from build123d import *

# Parameters (mm, degrees)
ELBOW_SECTION_SKETCH_210_290_R    = 145
ELBOW_SECTION_SKETCH_210_290_R_2  = 105
FLANGE_A_SKETCH_R                 = 105
FLANGE_A_360X360X50_DEPTH         = 50
FLANGE_START                      = -50
FLANGE_B_SKETCH_R                 = 105
FLANGE_B_360X360X50_DEPTH         = 50
EDGE_CHAMFER_5X45_A_SIZE          = 5
EDGE_CHAMFER_5X45_B_SIZE          = 5
FLANGE_B_BOLT_HOLES_SKETCH_R      = 15
FLANGE_B_BOLT_HOLES_30_DEPTH      = 50
FLANGE_B_COUNTERBORES_SKETCH_R    = 30
FLANGE_B_COUNTERBORES_60X10_DEPTH = 10
FLANGE_A_BOLT_HOLES_SKETCH_R      = 15
FLANGE_A_BOLT_HOLES_30_DEPTH      = 50
FLANGE_A_COUNTERBORES_SKETCH_R    = 30
FLANGE_A_COUNTERBORES_60X10_DEPTH = 10


with BuildPart() as part:
    # Elbow Body: sweep along a path in Elbow Path Sketch
    with BuildLine(Plane.XY) as elbow_body_path:
        Line((0, 0), (0, 150))
        ThreePointArc((0, 150), (76.152236891, 333.847763109), (260, 410))
        Line((260, 410), (410, 410))
    # Elbow Section Sketch Ø210-Ø290 → Elbow Body (sweep)
    with BuildSketch(Plane(origin=(410, 0, 0), x_dir=(0, 0, -1), z_dir=(1, 0, 0))):
        with Locations((0, 410)):
            Circle(ELBOW_SECTION_SKETCH_210_290_R)
        with Locations((0, 410)):
            Circle(ELBOW_SECTION_SKETCH_210_290_R_2, mode=Mode.SUBTRACT)
    sweep(path=elbow_body_path.line)

    # Flange A Sketch → Flange A 360x360x50 (add)
    with BuildSketch(Plane(origin=(410, 0, 0), x_dir=(0, 0, -1), z_dir=(1, 0, 0))):
        with BuildLine():
            Line((-160, 230), (160, 230))
            ThreePointArc((160, 230), (174.142135624, 235.857864376), (180, 250))
            Line((180, 250), (180, 570))
            ThreePointArc((180, 570), (174.142135624, 584.142135624), (160, 590))
            Line((160, 590), (-160, 590))
            ThreePointArc((-160, 590), (-174.142135624, 584.142135624), (-180, 570))
            Line((-180, 570), (-180, 250))
            ThreePointArc((-180, 250), (-174.142135624, 235.857864376), (-160, 230))
        make_face()
        with Locations((0, 410)):
            Circle(FLANGE_A_SKETCH_R, mode=Mode.SUBTRACT)
    extrude(amount=-FLANGE_A_360X360X50_DEPTH)

    # Flange B Sketch → Flange B 360x360x50 (add)
    with BuildSketch(Plane.XZ.offset(FLANGE_START)):
        with BuildLine():
            Line((-160, -180), (160, -180))
            ThreePointArc((160, -180), (174.142135624, -174.142135624), (180, -160))
            Line((180, -160), (180, 160))
            ThreePointArc((180, 160), (174.142135624, 174.142135624), (160, 180))
            Line((160, 180), (-160, 180))
            ThreePointArc((-160, 180), (-174.142135624, 174.142135624), (-180, 160))
            Line((-180, 160), (-180, -160))
            ThreePointArc((-180, -160), (-174.142135624, -174.142135624), (-160, -180))
        make_face()
        with Locations(Location((0, 0, 0), (0, 0, 180))):
            Circle(FLANGE_B_SKETCH_R, mode=Mode.SUBTRACT)
    extrude(amount=FLANGE_B_360X360X50_DEPTH)

    # Edge Chamfer 5x45 A
    edge_chamfer_5x45_a_edges = [part.edges().sort_by_distance(p)[0] for p in [
        (0, 0, 105),
    ]]
    chamfer(edge_chamfer_5x45_a_edges, length=EDGE_CHAMFER_5X45_A_SIZE)

    # Edge Chamfer 5x45 B
    edge_chamfer_5x45_b_edges = [part.edges().sort_by_distance(p)[0] for p in [
        (410, 410, 105),
    ]]
    chamfer(edge_chamfer_5x45_b_edges, length=EDGE_CHAMFER_5X45_B_SIZE)

    # Flange B Bolt Holes Sketch → Flange B Bolt Holes Ø30 (cut)
    with BuildSketch(Plane.XZ):
        with Locations(Location((-130, 130, 0), (0, 0, 270))):
            Circle(FLANGE_B_BOLT_HOLES_SKETCH_R)
        with Locations(Location((-130, -130, 0), (0, 0, 270))):
            Circle(FLANGE_B_BOLT_HOLES_SKETCH_R)
        with Locations(Location((130, -130, 0), (0, 0, 90))):
            Circle(FLANGE_B_BOLT_HOLES_SKETCH_R)
        with Locations(Location((130, 130, 0), (0, 0, 90))):
            Circle(FLANGE_B_BOLT_HOLES_SKETCH_R)
    extrude(amount=-FLANGE_B_BOLT_HOLES_30_DEPTH, mode=Mode.SUBTRACT)

    # Flange B Counterbores Sketch → Flange B Counterbores Ø60x10 (cut)
    with BuildSketch(Plane.XZ):
        with Locations(Location((-130, 130, 0), (0, 0, 270))):
            Circle(FLANGE_B_COUNTERBORES_SKETCH_R)
        with Locations(Location((-130, -130, 0), (0, 0, 270))):
            Circle(FLANGE_B_COUNTERBORES_SKETCH_R)
        with Locations(Location((130, -130, 0), (0, 0, 270))):
            Circle(FLANGE_B_COUNTERBORES_SKETCH_R)
        with Locations(Location((130, 130, 0), (0, 0, 270))):
            Circle(FLANGE_B_COUNTERBORES_SKETCH_R)
    extrude(amount=-FLANGE_B_COUNTERBORES_60X10_DEPTH, mode=Mode.SUBTRACT)

    # Flange A Bolt Holes Sketch → Flange A Bolt Holes Ø30 (cut)
    with BuildSketch(Plane(origin=(410, 0, 0), x_dir=(0, 0, -1), z_dir=(1, 0, 0))):
        with Locations((-130, 540)):
            Circle(FLANGE_A_BOLT_HOLES_SKETCH_R)
        with Locations((-130, 280)):
            Circle(FLANGE_A_BOLT_HOLES_SKETCH_R)
        with Locations(Location((130, 280, 0), (0, 0, 180))):
            Circle(FLANGE_A_BOLT_HOLES_SKETCH_R)
        with Locations(Location((130, 540, 0), (0, 0, 180))):
            Circle(FLANGE_A_BOLT_HOLES_SKETCH_R)
    extrude(amount=-FLANGE_A_BOLT_HOLES_30_DEPTH, mode=Mode.SUBTRACT)

    # Flange A Counterbores Sketch → Flange A Counterbores Ø60x10 (cut)
    with BuildSketch(Plane(origin=(410, 0, 0), x_dir=(0, 0, -1), z_dir=(1, 0, 0))):
        with Locations((-130, 540)):
            Circle(FLANGE_A_COUNTERBORES_SKETCH_R)
        with Locations((130, 540)):
            Circle(FLANGE_A_COUNTERBORES_SKETCH_R)
        with Locations((-130, 280)):
            Circle(FLANGE_A_COUNTERBORES_SKETCH_R)
        with Locations((130, 280)):
            Circle(FLANGE_A_COUNTERBORES_SKETCH_R)
    extrude(amount=-FLANGE_A_COUNTERBORES_60X10_DEPTH, mode=Mode.SUBTRACT)


solid = part.part
Verification items for the finished model (mm, model axes). A direction names the side the tool comes from. Give positions to 0.01 mm unless a question says otherwise; leave off trailing zeros. Loops run counter-clockwise (first coordinate to the right, second up) from the corner with the lowest first, then second, coordinate; pieces in that order, holes last. Notation, with made-up numbers: (-33, 33.5) - (-25, 33.5) arc R27 cw to (-25, 58.5) - close; hole circle Ø1 at (14.5, -27.5). An arc over 180 degrees is marked (long way). Write item = value, one per line. Start each with the question number.
Q1. Tool access check on faces 4 (the face through (360, 533, 83)), 5 (the face through (115.128, 29.72, -131.953)), 6 (the face through (180, 25, -2)). Record the directions out of +Z, -Z, +X, -X, +Y, -Y that give a thin tool (end or side, any length) a straight path to the whole face; none if there is none.
Q2. Cross-section at D-D, the plane x = 130. State how many separate pieces and enclosed holes the cut face has, and give its area (3 significant figures).
Q3. Depth check by flat-ended pin: P1, Ø10, axis at y = 296.5, z = -12, coming from the -X side; P2, Ø6, axis at x = 69, y = 199.5, coming from the +Z side; P3, Ø1, axis at y = 101.5, z = -29, coming from the +X side. Enter the tip coordinate at first touch or a pass-through.
Q4. Mould release check, pull along Y, two halves, no side actions. Record for faces 1 (the face through (380.28, 554.643, -133.252)), 2 (the face through (-115.128, 29.72, 131.953)), 3 (the face through (-83, 0, 83)): released by +Y, released by -Y, zero draft, split by the parting line, or undercut.
Q5. Thickness scan on line 1 (Y direction, x = 403.5, z = -130); line 2 (Y direction, x = 388, z = 130); line 3 (X direction, y = 7.25, z = -130). Record the ranges inside material, lowest first.
Q6. Cross-section at B-B, the plane y = 72. Enter the section's corners in (x, z), and give its area (3 significant figures).
Q7. Cross-section at C-C, the plane x = 303. Enter the section's corners in (y, z), and give its area (3 significant figures).
Q8. Cross-section at A-A, the plane z = 0. Enter the section's corners in (x, y), and give its area (3 significant figures).
Answer key:
q1.face_4 = none
q1.face_5 = -Y
q1.face_6 = +Z, -Z, +X, -Y
q2.separate_pieces = 3
q2.enclosed_holes = 1
q2.area = 71,600 mm^2
q3.P1 = -118.99
q3.P2 = 132.14
q3.P3 = 142.17
q4.face_1 = undercut
q4.face_2 = zero draft
q4.face_3 = released by -Y
q5.line_1 = 230 to 250, 310 to 510, 570 to 590
q5.line_2 = 230 to 265, 295 to 525, 555 to 590
q5.line_3 = -180 to -160, -100 to 100, 160 to 180
q6.outline = circle Ø290 at (0, 0); hole circle Ø210 at (0, 0)
q6.area = 31,400 mm^2
q7.outline = circle Ø290 at (410, 0); hole circle Ø210 at (410, 0)
q7.area = 31,400 mm^2
q8.outline = (-180, 0) - (-110, 0) - (-105, 5) - (-105, 150) arc R365 cw to (260, 515) - (405, 515) - (410, 520) - (410, 590) - (360, 590) - (360, 555) - (260, 555) arc R405 ccw to (-145, 150) - (-145, 50) - (-180, 50) - close; (105, 5) - (110, 0) - (180, 0) - (180, 50) - (145, 50) - (145, 150) arc R115 cw to (260, 265) - (360, 265) - (360, 230) - (410, 230) - (410, 300) - (405, 305) - (260, 305) arc R155 ccw to (105, 150) - close
q8.area = 63,600 mm^2
